Read the model definition and answer for the solid it produces. Units are mm, in the model's axes. Face numbers are marked on the shaded views. A direction names the side the tool comes from. Coordinates: 2 decimals unless noted, no trailing zeros. Loops run counter-clockwise (first coordinate to the right, second up) from the corner with the lowest first, then second, coordinate; pieces in that order, holes last. Notation, with made-up numbers: (63.25, 39.25) - (76.25, 39.25) arc R16 cw to (76.25, 44.25) - close; hole circle Ø8 at (24.25, -34). An arc over 180 degrees is marked (long way). Use one line per item in the form item = value.
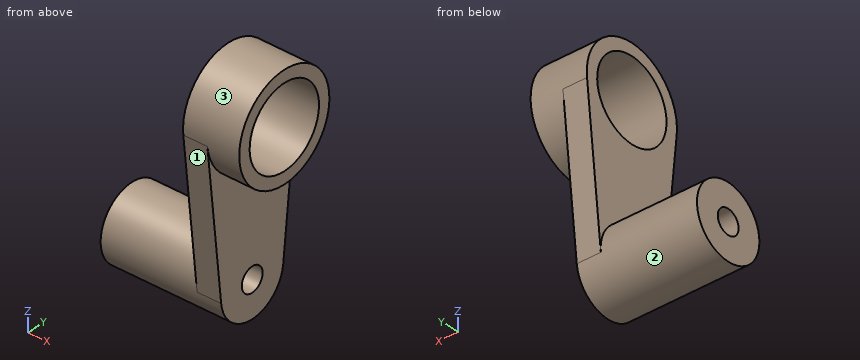
from build123d import *

# Parameters (mm, degrees)
HUB_AND_POST_PROFILE_SKETCH_R   = 13
HUB_AND_POST_PROFILE_SKETCH_R_2 = 10
HUB_RING_26X_20_DEPTH           = 14
SKETCH1_3_R                     = 9
PIN_POST_18_DEPTH               = 24
ARM_WEB_SKETCH_R                = 9
ARM_WEB_6MM_DEPTH               = 6
PIN_HOLE_SKETCH_R               = 3
PIN_HOLE_6_DEPTH                = 37


with BuildPart() as part:
    # Hub and Post Profile Sketch → Hub Ring _26x_20 (new body)
    with BuildSketch(Plane(origin=(0, 0, 0), x_dir=(0, 0, -1), z_dir=(1, 0, 0))):
        Circle(HUB_AND_POST_PROFILE_SKETCH_R)
        Circle(HUB_AND_POST_PROFILE_SKETCH_R_2, mode=Mode.SUBTRACT)
    extrude(amount=HUB_RING_26X_20_DEPTH)



with BuildPart() as body_2:
    # Sketch1_3 → Pin Post _18 (new body)
    with BuildSketch(Plane(origin=(0, 0, 0), x_dir=(0, 0, -1), z_dir=(1, 0, 0))):
        with Locations((38, 0)):
            Circle(SKETCH1_3_R)
    extrude(amount=-PIN_POST_18_DEPTH)


with BuildPart() as part_1:
    add(part.part)

    add(body_2.part)  # Arm Web 6mm merges body 2
    # Arm Web Sketch → Arm Web 6mm (add)
    with BuildSketch(Plane(origin=(0, 0, 0), x_dir=(0, 0, -1), z_dir=(1, 0, 0))):
        with BuildLine():
            Line((38.947368421, 8.949999613), (1.368421053, 12.927777219))
            ThreePointArc((1.368421053, 12.927777219), (9.664095242, 8.695128703), (13, 0))
            ThreePointArc((13, 0), (9.664095242, -8.695128703), (1.368421053, -12.927777219))
            Line((1.368421053, -12.927777219), (38.947368421, -8.949999613))
            ThreePointArc((38.947368421, -8.949999613), (29, 0), (38.947368421, 8.949999613))
        make_face()
        with Locations(Location((38, 0, 0), (0, 0, 276.042328419))):
            Circle(ARM_WEB_SKETCH_R)
    extrude(amount=ARM_WEB_6MM_DEPTH)

    # Pin Hole Sketch → Pin Hole _6 (cut)
    with BuildSketch(Plane(origin=(6, 0, 0), x_dir=(0, 0, -1), z_dir=(1, 0, 0))):
        with Locations((38, 0)):
            Circle(PIN_HOLE_SKETCH_R)
    extrude(amount=-PIN_HOLE_6_DEPTH, mode=Mode.SUBTRACT)


solid = part_1.part
Item 1: The part is cut by section C-C on y = 0. Give the vertices of the cut face in (x, z), plus the area to 3 significant figures.
Results below:
outline = (-24, -47) - (6, -47) - (6, -41) - (-24, -41) - close; (-24, -35) - (6, -35) - (6, -13) - (14, -13) - (14, -10) - (0, -10) - (0, -29) - (-24, -29) - close; (0, 10) - (14, 10) - (14, 13) - (0, 13) - close
area = 540 mm²
Item 2: Find the intervals of material crossed by L1, parallel to Y at x = -9.5, z = -38; L2, parallel to X at y = 1, z = -11; L3, parallel to X at y = 8.5, z = -13.5, in increasing order.
Results below:
L1 = -9 to -3, 3 to 9
L2 = 0 to 14
L3 = 0 to 6
Item 3: The part is cut by section B-B on y = 4.5. Give the vertices of the cut face in (x, z).
Results below:
outline = (-24, -45.79) - (6, -45.79) - (6, -12.2) - (14, -12.2) - (14, -8.93) - (0, -8.93) - (0, -30.21) - (-24, -30.21) - close; (0, 8.93) - (14, 8.93) - (14, 12.2) - (0, 12.2) - close
Item 4: The part is cut by section D-D on x = 9.5. Give the vertices of the cut face in (y, z), plus the area to 3 significant figures.
Results below:
outline = circle Ø26 at (0, 0); hole circle Ø20 at (0, 0)
area = 217 mm²
Item 5: Each of these flat-tipped pins is pushed along its axis until it touches: P1, Ø1.5, axis at y = -4, z = -9, coming from the +X side; P2, Ø12, axis at x = -5.5, z = -8, coming from the -Y side; P3, Ø2, axis at x = -3.5, z = -30, coming from the -Y side; P4, Ø3, axis at x = -12, y = 2, coming from the -Z side. Where does it stop, or does it pass through?
Results below:
P1 = 14
P2 = -12.48
P3 = -5.66
P4 = -46.99
Item 6: Which of the six approach directions +Z, -Z, +X, -X, +Y, -Y give full straight-line access (tool end or side, diameter ignored) to the marked faces 1, 2 and 3?
Results below:
face_1 = -Z, +X, -X, -Y
face_2 = -X
face_3 = +X
Item 7: The part is cut by section A-A on z = 0. Give the vertices of the cut face in (x, y).
Results below:
outline = (0, -13) - (14, -13) - (14, -10) - (0, -10) - close; (0, 10) - (14, 10) - (14, 13) - (0, 13) - close
